Can you work these out from the model? Positions are in its coordinate system, mm. A direction names the side the tool comes from. Give positions to 0.01 mm unless a question says otherwise; leave off trailing zeros. Order: outer loops, then holes, each group sorted by start corner. A loop starts at its lowest first (then second) coordinate and runs counter-clockwise, first axis right, second up. Notation, with made-up numbers: M 32,49.5 L 69,49.5 A19 ccw 69,81.5 Z; hole C -5.5,-30 d9. An arc over 180 degrees is marked long. Answer as a JSON object with one key per item and string values.
```python
from build123d import *

# Parameters (mm, degrees)
BOSS_EXTRUDE1_DEPTH = 1681
SKETCH3_W           = 250
SKETCH3_H           = 146.5
CUT_EXTRUDE1_DEPTH  = 16


with BuildPart() as part:
    # Sketch1 → Boss-Extrude1 (new body)
    with BuildSketch(Plane.XY):
        with BuildLine():
            Line((0, 0), (250, 0))
            Line((250, 0), (250, 14))
            Line((250, 14), (142.5, 14))
            ThreePointArc((142.5, 14), (133.307611845, 17.807611845), (129.5, 27))
            Line((129.5, 27), (129.5, 223))
            ThreePointArc((129.5, 223), (133.307611845, 232.192388155), (142.5, 236))
            Line((142.5, 236), (250, 236))
            Line((250, 236), (250, 250))
            Line((250, 250), (0, 250))
            Line((0, 250), (0, 236))
            Line((0, 236), (107.5, 236))
            ThreePointArc((107.5, 236), (116.692388155, 232.192388155), (120.5, 223))
            Line((120.5, 223), (120.5, 27))
            ThreePointArc((120.5, 27), (116.692388155, 17.807611845), (107.5, 14))
            Line((107.5, 14), (0, 14))
            Line((0, 14), (0, 0))
        make_face()
    extrude(amount=BOSS_EXTRUDE1_DEPTH)

    # Sketch3 → Cut-Extrude1 (cut)
    with BuildSketch(Plane(origin=(0, 0, 0), x_dir=(-1, 0, 0), z_dir=(0, -1, 0))):
        with Locations((-125, -73.25)):
            Rectangle(SKETCH3_W, SKETCH3_H)
        with Locations((-125, -1607.75)):
            Rectangle(SKETCH3_W, SKETCH3_H)
    extrude(amount=-CUT_EXTRUDE1_DEPTH, mode=Mode.SUBTRACT)


solid = part.part
```
1) I want a section at C-C on y = 100.5. Write out the boundary of the cut face in (x, z), and give its area (3 significant figures).
Results found:
{"outline": "M 120.5,0 L 129.5,0 L 129.5,1681 L 120.5,1681 Z", "area": "15,100 mm²"}
2) Thinking about a two-plate mould opening in Y: for faces 1 (the face through (124, 203, 1681)), 2 (the face through (55, 14, 831)), 3 (the face through (127, 250, 829)), which applies, pulls with the +Y half, pulls with the -Y half, needs draft (parallel to the pull), parting line crosses it, or undercut?
Results found:
{"face 1": "needs draft", "face 2": "undercut", "face 3": "pulls with the +Y half"}
3) I need wall thicknesses on L1, parallel to Y at x = 145.5, z = 568; L2, parallel to X at y = 96, z = 1406.5; L3, parallel to Z at x = 232, y = 12.5. Which ranges of each line are inside material? Lowest first, please.
Results found:
{"L1": "y = 0 to 14, 236 to 250", "L2": "x = 120.5 to 129.5", "L3": "z = 146.5 to 1534.5"}
4) I want a section at B-B on z = 799.5. Write out the boundary of the cut face in (x, y).
Results found:
{"outline": "M 0,0 L 250,0 L 250,14 L 142.5,14 A13 cw 129.5,27 L 129.5,223 A13 cw 142.5,236 L 250,236 L 250,250 L 0,250 L 0,236 L 107.5,236 A13 cw 120.5,223 L 120.5,27 A13 cw 107.5,14 L 0,14 Z"}
5) For faces 4 (the face through (120.5, 126, 829)), 5 (the face through (123, 0, 831)), 6 (the face through (129.5, 124, 829)), which set-ups out of +Z, -Z, +X, -X, +Y, -Y let a thin tool reach every point of the face, with its end or its side?
Results found:
{"face 4": "+Z, -Z, -X", "face 5": "+Z, -Z, +X, -X, -Y", "face 6": "+Z, -Z, +X"}
6) I want a section at A-A on x = 78.5. Write out the boundary of the cut face in (y, z), and give its area (3 significant figures).
Results found:
{"outline": "M 0,146.5 L 14,146.5 L 14,1534.5 L 0,1534.5 Z; M 236,0 L 250,0 L 250,1681 L 236,1681 Z", "area": "43,000 mm²"}
7) I'm going to push flat-ended pins straight in: pin 1 Ø8 at (x, y) = (111.5, 8.5) entering from -Z; pin 2 Ø3 at (y, z) = (108.5, 540.5) entering from +X; pin 3 Ø12 at (x, z) = (195, 200.5) entering from -Y; pin 4 Ø8 at (x, y) = (86, 9.5) entering from +Z. Where does each tip first touch, or does it pass through?
Results found:
{"pin 1": "stops at z = 146.5", "pin 2": "stops at x = 129.5", "pin 3": "stops at y = 0", "pin 4": "stops at z = 1534.5"}
